Could you check a few things on this drawing? It's one solid part, dimensions in mm from its lowest x, y, z. Round coordinates to 2 decimals unless told otherwise and drop trailing zeros. Write each loop counter-clockwise with the first axis right and the second up, starting at its lowest first coordinate (ties: lowest second). Pieces come first, ordered by that corner, then holes. Notation, with made-up numbers: (16, 31.5) -> (32, 31.5) arc R22 cw to (32, 45.5) -> close; hole circle Ø2 at (76, -39.75). An arc over 180 degrees is marked (long way). Answer in a Markdown table with one row per item.
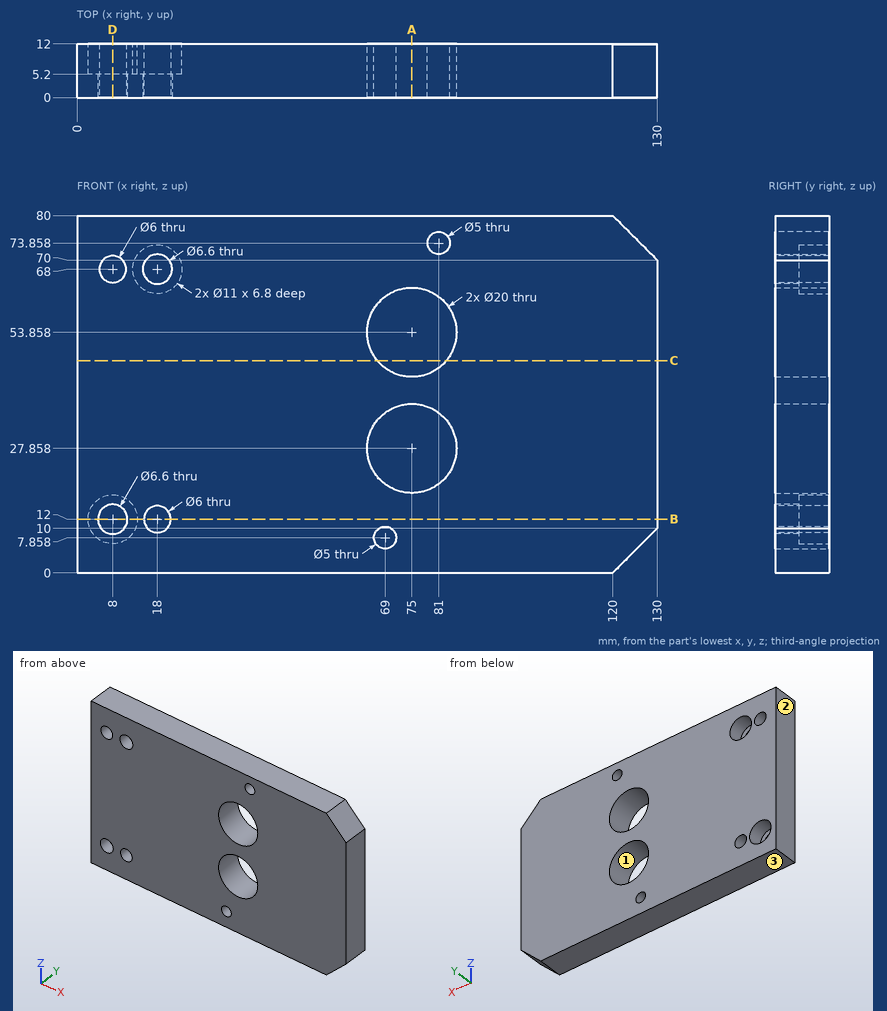
1) I want a section at D-D, the plane x = 8. List the corners of the cut face in (y, z) for me, and give its area (3 significant figures).
Response:
| item | result |
|---|---|
| outline | (0, 0) -> (12, 0) -> (12, 6.5) -> (5.2, 6.5) -> (5.2, 8.7) -> (0, 8.7) -> close; (0, 15.3) -> (5.2, 15.3) -> (5.2, 17.5) -> (12, 17.5) -> (12, 65) -> (0, 65) -> close; (0, 71) -> (12, 71) -> (12, 80) -> (0, 80) -> close |
| area | 779 mm^2 |
2) We'd pull the mould along Z, two halves only. Please class the marked faces 1, 2 and 3: +Z half, -Z half, draft (parallel to the pull), parting line (faces both ways), or undercut.
Response:
| item | result |
|---|---|
| face 1 | undercut |
| face 2 | draft |
| face 3 | -Z half |
3) I need wall thicknesses on line 1 (X direction, y = 3.5, z = 68); line 2 (X direction, y = 10.75, z = 12); line 3 (Z direction, x = 81, y = 5). Which ranges of each line are inside material? Lowest first, please. Write a range as [from, to].
Response:
| item | result |
|---|---|
| line 1 | x = [0, 5], [11, 14.7], [21.3, 130] |
| line 2 | x = [0, 2.5], [13.5, 15], [21, 130] |
| line 3 | z = [0, 19.86], [35.86, 45.86], [61.86, 71.36], [76.36, 80] |
4) I want a section at B-B, the plane z = 12. List the corners of the cut face in (x, y) for me.
Response:
| item | result |
|---|---|
| outline | (0, 0) -> (4.7, 0) -> (4.7, 5.2) -> (2.5, 5.2) -> (2.5, 12) -> (0, 12) -> close; (11.3, 0) -> (15, 0) -> (15, 12) -> (13.5, 12) -> (13.5, 5.2) -> (11.3, 5.2) -> close; (21, 0) -> (130, 0) -> (130, 12) -> (21, 12) -> close |
5) I want a section at C-C, the plane z = 47.5. List the corners of the cut face in (x, y) for me, and give its area (3 significant figures).
Response:
| item | result |
|---|---|
| outline | (0, 0) -> (67.28, 0) -> (67.28, 12) -> (0, 12) -> close; (82.72, 0) -> (130, 0) -> (130, 12) -> (82.72, 12) -> close |
| area | 1,370 mm^2 |
6) I want a section at A-A, the plane x = 75. List the corners of the cut face in (y, z) for me.
Response:
| item | result |
|---|---|
| outline | (0, 0) -> (12, 0) -> (12, 17.86) -> (0, 17.86) -> close; (0, 37.86) -> (12, 37.86) -> (12, 43.86) -> (0, 43.86) -> close; (0, 63.86) -> (12, 63.86) -> (12, 80) -> (0, 80) -> close |
7) For pin 1 (4.5 mm diameter, centred on x = 69, z = 7.86, fed in from -Y); pin 2 (5.5 mm diameter, centred on x = 10, z = 12.5, fed in from +Y), each with a flat end and sliding along its axis, tell me the tip position at first contact or that it passes through.
Response:
| item | result |
|---|---|
| pin 1 | passes through |
| pin 2 | stops at y = 5.2 |
